```python
from build123d import *

# Parameters (mm, degrees)
EXTRUDE_1_DEPTH      = 5.5
EXTRUDE_1_DEPTH_BACK = 5.5
SKETCH_2_W           = 108
SKETCH_2_H           = 22
CUT_EXTRUDE_1_DEPTH  = 11
SKETCH_4_W           = 9
SKETCH_4_H           = 10
CUT_EXTRUDE_2_DEPTH  = 11


with BuildPart() as part:
    # 草图1 → 凸台-拉伸1 (new, two sides: drawn at the far end of the back side and taken through both)
    with BuildSketch(Plane.XY.offset(-EXTRUDE_1_DEPTH_BACK)):
        with BuildLine():
            Line((0, 0), (27, 0))
            Line((27, 0), (27, 1))
            Line((27, 1), (6.99, 1))
            ThreePointArc((6.99, 1), (6.636446609, 1.146446609), (6.49, 1.5))
            Line((6.49, 1.5), (6.49, 1.724666059))
            Line((6.49, 1.724666059), (4.63, 1.887394973))
            ThreePointArc((4.63, 1.887394973), (5.459499899, 4.491284383), (3.833170563, 6.6875))
            ThreePointArc((3.833170563, 6.6875), (2.5, 4.5), (1.166829437, 6.6875))
            ThreePointArc((1.166829437, 6.6875), (0.515533844, 6.249865346), (0, 5.658312395))
            Line((0, 5.658312395), (0, 0))
        make_face()
    extrude(amount=EXTRUDE_1_DEPTH + EXTRUDE_1_DEPTH_BACK)

    # 草图2 → 切除-拉伸1 (cut)
    with BuildSketch(Plane(origin=(0, 0, 0), x_dir=(1, 0, 0), z_dir=(0, 1, 0))):
        Rectangle(SKETCH_2_W, SKETCH_2_H)
        with BuildLine():
            Line((0, 5.5), (0, -5.5))
            Line((0, -5.5), (21.5, -5.5))
            ThreePointArc((21.5, -5.5), (27, 0), (21.5, 5.5))
            Line((21.5, 5.5), (0, 5.5))
        make_face(mode=Mode.SUBTRACT)
    extrude(amount=CUT_EXTRUDE_1_DEPTH, mode=Mode.SUBTRACT)

    # 草图4 → 切除-拉伸2 (cut)
    with BuildSketch(Plane(origin=(0, 0, 0), x_dir=(0, 0, -1), z_dir=(1, 0, 0))):
        with Locations((0, 6)):
            Rectangle(SKETCH_4_W, SKETCH_4_H)
    extrude(amount=CUT_EXTRUDE_2_DEPTH, mode=Mode.SUBTRACT)

    # 草图3 → 切除-旋转1 (revolve, cut)
    with BuildSketch(Plane.XY, mode=Mode.PRIVATE) as cut_revolve_1_sk:
        Polygon((7.5, 1), (10.1, 1), (9.1, 0), (7.5, 0), align=None)
    revolve(cut_revolve_1_sk.sketch.rotate(Axis((7.5, 0, 0), (0, 1, 0)), 270), axis=Axis((7.5, 0, 0), (0, 1, 0)), mode=Mode.SUBTRACT)

    # 草图5 → 切除-旋转2 (revolve, cut)
    with BuildSketch(Plane.XY, mode=Mode.PRIVATE) as cut_revolve_2_sk:
        Polygon((20.5, 1), (23.1, 1), (22.1, 0), (20.5, 0), align=None)
    revolve(cut_revolve_2_sk.sketch.rotate(Axis((20.5, 0, 0), (0, 1, 0)), 270), axis=Axis((20.5, 0, 0), (0, 1, 0)), mode=Mode.SUBTRACT)


solid = part.part
```
Here's how the part is built. I have some questions about the finished solid (model axes, mm). A direction names the side the tool comes from. Coordinates: 2 decimals unless noted, no trailing zeros. Loops run counter-clockwise (first coordinate to the right, second up) from the corner with the lowest first, then second, coordinate; pieces in that order, holes last. Notation, with made-up numbers: (18.5, 63.5) - (59.5, 63.5) arc R14 cw to (59.5, 78.5) - close; hole circle Ø5 at (47, 9). An arc over 180 degrees is marked (long way). Return JSON: item names as keys, results as strings. Group by question number.
Item 1: Will these pins go through, and if not, where does the flat tip stop? P1, Ø2, axis at y = 5, z = -4, coming from the +X side; P2, Ø2, axis at x = 23.5, y = 0.5, coming from the +Z side; P3, Ø2, axis at x = 5, z = -4, coming from the +Y side.
Item 2: If we section it at B-B on x = 7.5: Write out the boundary of the cut face in (y, z).
Item 3: If we section it at D-D on y = 6: Write out the boundary of the cut face in (x, z), and give its area (3 significant figures).
Item 4: On a 3-axis mill with a long thin cutter (end or side, diameter ignored), from which of +Z, -Z, +X, -X, +Y, -Y can I reach the whole of each face in a straight line? I mean faces 4 (the face through (27, 0.5, 0.1)), 5 (the face through (3, 3, -4.5)), 6 (the face through (14, 1, 0)), 7 (the face through (5.573, 1.805, 4.993)). Say none if no direction works.
Item 5: We'd pull the mould along Y, two halves only. Please class faces 1 (the face through (0, 0.4, -0.1)), 2 (the face through (13, 0, 0)), 3 (the face through (2.5, 4.5, 5)): +Y half, -Y half, draft (parallel to the pull), parting line (faces both ways), or undercut.
Item 6: I need wall thicknesses on line 1 (X direction, y = 6, z = 5.3); line 2 (Y direction, x = 1.25, z = 2.5). Which ranges of each line are inside material? Lowest first, please. Write a range as from..to.
Item 7: If we section it at C-C on y = 3.25: Write out the boundary of the cut face in (x, z), and give its area (3 significant figures).
Item 8: If we section it at A-A on z = 0: Write out the boundary of the cut face in (x, y).
Calculated:
{
 "1": {"P1": "stops at x = 5.5", "P2": "stops at z = 5.41", "P3": "stops at y = 6.52"},
 "2": {"outline": "(0, -5.5) - (1, -5.5) - (1, -2.6) - (0, -1.6) - close; (0, 1.6) - (1, 2.6) - (1, 5.5) - (0, 5.5) - close"},
 "3": {"outline": "(0.26, -5.5) - (1, -5.5) - (1, -4.5) - (0.26, -4.5) - close; (0.26, 4.5) - (1, 4.5) - (1, 5.5) - (0.26, 5.5) - close; (4, -5.5) - (4.74, -5.5) - (4.74, -4.5) - (4, -4.5) - close; (4, 4.5) - (4.74, 4.5) - (4.74, 5.5) - (4, 5.5) - close", "area": "2.94 mm^2"},
 "4": {"face 4": "+X, +Y, -Y", "face 5": "+X, -X, +Y", "face 6": "+X, +Y", "face 7": "+Z, -Z, +X"},
 "5": {"face 1": "draft", "face 2": "-Y half", "face 3": "undercut"},
 "6": {"line 1": "x = 0.26..1, 4..4.74", "line 2": "y = 0..1"},
 "7": {"outline": "(0, -5.5) - (5.4, -5.5) - (5.4, -4.5) - (0, -4.5) - close; (0, 4.5) - (5.4, 4.5) - (5.4, 5.5) - (0, 5.5) - close", "area": "10.8 mm^2"},
 "8": {"outline": "(0, 0) - (5.9, 0) - (4.9, 1) - (0, 1) - close; (9.1, 0) - (18.9, 0) - (17.9, 1) - (10.1, 1) - close; (22.1, 0) - (27, 0) - (27, 1) - (23.1, 1) - close"}
}
